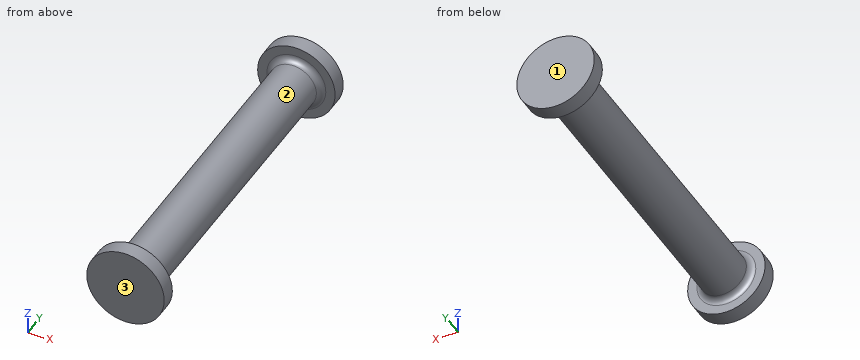
```python
from build123d import *

# Parameters (mm, degrees)
FILLET_1_R = 2


with BuildPart() as part:
    # 草图1 → 旋转2 (revolve)
    with BuildSketch(Plane.XY, mode=Mode.PRIVATE) as revolve_2_sk:
        Polygon((0, -50), (0, 60), (12.5, 60), (12.5, 55), (7.5, 55), (7.5, -45), (12.5, -45), (12.5, -50), align=None)
    revolve(revolve_2_sk.sketch.rotate(Axis((0, -50, 0), (0, 1, 0)), 90), axis=Axis((0, -50, 0), (0, 1, 0)))

    # 圆角1
    fillet_1_edges = [part.edges().sort_by_distance(p)[0] for p in [
        (0, -45, 7.5),
        (0, 55, 7.5),
    ]]
    fillet(fillet_1_edges, radius=FILLET_1_R)


solid = part.part
```
Input: part model. Units: mm. Frame: model coordinates. Face numbers are marked on the shaded views. Coordinates: 2 decimals unless noted, no trailing zeros. Write each loop counter-clockwise with the first axis right and the second up, starting at its lowest first coordinate (ties: lowest second). Pieces come first, ordered by that corner, then holes.
1) Material intervals for line 1 along Y through (x, z) = (-10, -1.75); line 2 along Y through (x, z) = (6, -5.25); line 3 along X through (y, z) = (-36.5, 0.25), sorted ascending.
2) Section D-D on y = 34.5. Output: boundary loops of the cut face in (x, z).
3) Section A-A on x = 0. Output: boundary loops of the cut face in (y, z), and give its area (3 significant figures).
4) Mould query, pull axis Y, two halves, no side actions, for the marked faces 1, 2 and 3. Classes: pulls with the +Y half, pulls with the -Y half, needs draft (parallel to the pull), parting line crosses it, or undercut.
5) Pin query (flat end, axial travel): pin 1 Ø1 at (y, z) = (-1, -8.5) entering from +X; pin 2 Ø5 at (y, z) = (-5.5, 5.5) entering from -X; pin 3 Ø2 at (y, z) = (1.5, 4) entering from +X; pin 4 Ø1.5 at (x, y) = (5.5, 45.5) entering from -Z. Return the tip coordinate at first contact, or that it passes through.
6) Section C-C on z = 10.75. Output: boundary loops of the cut face in (x, y).
7) Section B-B on z = 0. Output: boundary loops of the cut face in (x, y).
Check result:
1. line 1: y = -50 to -45, 55 to 60
1. line 2: y = -50 to -44.29, 54.29 to 60
1. line 3: x = -7.5 to 7.5
2. outline: circle Ø15 at (0, 0)
3. outline: (-50, -12.5) - (-45, -12.5) - (-45, -9.5) arc R2 cw to (-43, -7.5) - (53, -7.5) arc R2 cw to (55, -9.5) - (55, -12.5) - (60, -12.5) - (60, 12.5) - (55, 12.5) - (55, 9.5) arc R2 cw to (53, 7.5) - (-43, 7.5) arc R2 cw to (-45, 9.5) - (-45, 12.5) - (-50, 12.5) - close
3. area: 1,750 mm2
4. face 1: pulls with the +Y half
4. face 2: undercut
4. face 3: pulls with the -Y half
5. pin 1: passes through
5. pin 2: stops at x = -6.87
5. pin 3: stops at x = 6.87
5. pin 4: stops at z = -5.8
6. outline: (-6.38, -50) - (6.38, -50) - (6.38, -45) - (-6.38, -45) - close; (-6.38, 55) - (6.38, 55) - (6.38, 60) - (-6.38, 60) - close
7. outline: (-12.5, -50) - (12.5, -50) - (12.5, -45) - (9.5, -45) arc R2 cw to (7.5, -43) - (7.5, 53) arc R2 cw to (9.5, 55) - (12.5, 55) - (12.5, 60) - (-12.5, 60) - (-12.5, 55) - (-9.5, 55) arc R2 cw to (-7.5, 53) - (-7.5, -43) arc R2 cw to (-9.5, -45) - (-12.5, -45) - close
